from build123d import *

# Parameters (mm, degrees)
HOUSING_REVOLVE_270DEG_ANGLE = 270


with BuildPart() as part:
    # Stepped Housing Profile → Housing Revolve 270deg (revolve)
    with BuildSketch(Plane.XY):
        Polygon((0, 40), (0, 10), (120, 10), (120, 20), (64, 20), (64, 40), (96, 40), (96, 65), (128, 65), (128, 75), (160, 75), (160, 85), (120, 85), (120, 70), (80, 70), (80, 55), (40, 55), (40, 40), align=None)
    revolve(axis=Axis((0, 0, 0), (1, 0, 0)), revolution_arc=HOUSING_REVOLVE_270DEG_ANGLE)


solid = part.part
Build history of the part. All positions in model axes, mm. A direction names the side the tool comes from. Give positions to 0.01 mm unless a question says otherwise; leave off trailing zeros. Order: outer loops, then holes, each group sorted by start corner. A loop starts at its lowest first (then second) coordinate and runs counter-clockwise, first axis right, second up. Notation, with made-up numbers: M 20.5,-34.5 L 56.5,-34.5 A25 ccw 56.5,-16.5 Z; hole C 44.25,-38 d4. An arc over 180 degrees is marked long. Use one line per item in the form item = value.
1) Saw through at B-B (y = -47.5). Give the cut face in (x, z).
Calculated:
outline = M 40,-27.73 L 80,-27.73 L 80,-51.42 L 120,-51.42 L 120,-70.49 L 160,-70.49 L 160,-58.04 L 128,-58.04 L 128,-44.37 L 96,-44.37 L 96,44.37 L 128,44.37 L 128,58.04 L 160,58.04 L 160,70.49 L 120,70.49 L 120,51.42 L 80,51.42 L 80,27.73 L 40,27.73 Z
2) Two-plate mould, pull along Z, no slides. Class faces 6 (the face through (64, -17, 18)), 7 (the face through (62, 37, 0)), 8 (the face through (40, -29, 29)): released by +Z, released by -Z, zero draft, split by the parting line, or undercut.
Calculated:
face_6 = undercut
face_7 = released by -Z
face_8 = zero draft
3) Probe probe 1 along Y at (x, z) = (73, 0.5); probe 2 along X at (y, z) = (9, 12.5); probe 3 along X at (y, z) = (-70.5, 3.5). List the from-to ranges inside material, lowest first.
Calculated:
probe_1 = -55 to -40, -19.99 to -9.99, 9.99 to 19.99, 40 to 55
probe_2 = 0 to 120
probe_3 = 120 to 128
4) Saw through at A-A (z = -67.5). Give the cut face in (x, y).
Calculated:
outline = M 80,-18.54 L 120,-18.54 L 120,-51.66 L 160,-51.66 L 160,-32.69 L 128,-32.69 L 128,0 L 80,0 Z
5) Tool access for faces 1 (the face through (0, -9, 9)), 2 (the face through (62, 0, -37)), 3 (the face through (160, -56, 51)), 4 (the face through (99.72, -47.84, 51.1)), 5 (the face through (80.22, -27.34, 29.2)): list every direction of +Z, -Z, +X, -X, +Y, -Y with a clear straight run to the whole face (end or side of a thin tool).
Calculated:
face_1 = +Z, -Z, -X, +Y, -Y
face_2 = -Z, +X, -X, +Y
face_3 = +Z, -Z, +X, +Y, -Y
face_4 = -X
face_5 = +X
6) Saw through at D-D (z = -34). Give the cut face in (x, y), plus the area to 3 significant figures.
Calculated:
outline = M 0,-21.07 L 40,-21.07 L 40,-43.23 L 80,-43.23 L 80,-61.19 L 120,-61.19 L 120,-77.9 L 160,-77.9 L 160,-66.85 L 128,-66.85 L 128,-55.4 L 96,-55.4 L 96,-21.07 L 64,-21.07 L 64,0 L 0,0 Z
area = 3,550 mm2
7) Saw through at C-C (x = 131). Give the cut face in (y, z).
Calculated:
outline = M 0,-85 L 0,-75 A75 cw long 75,0 L 85,0 A85 ccw long Z
8) Drop flat-ended pins along their axis: pin 1 (1.5 mm diameter, centred on x = 142.5, z = 43.5, fed in from +Y); pin 2 (5 mm diameter, centred on x = 108, y = 14, fed in from -Z); pin 3 (2 mm diameter, centred on x = 106, z = -49.5, fed in from +Y). Give the stop position or say it passes through.
Calculated:
pin_1 = 73.47
pin_2 = 0
pin_3 = -40.92
